The figure shows three views and two pictorial views of one solid part (mm, origin at its lowest corner). Answer the questions. Coordinates: 2 decimals unless noted, no trailing zeros. Order: outer loops, then holes, each group sorted by start corner. A loop starts at its lowest first (then second) coordinate and runs counter-clockwise, first axis right, second up.
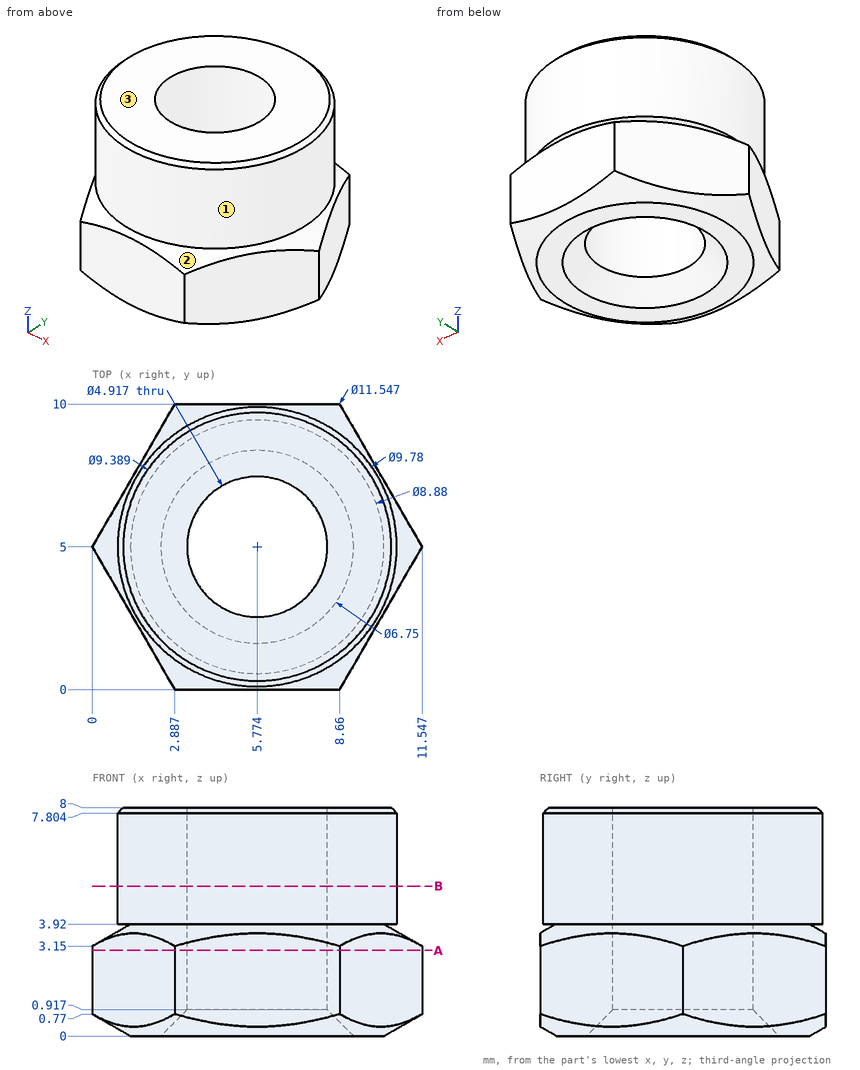
1) Straight lines are drawn through the part: probe 1 along X at (y, z) = (5.75, 3.5) (1 decimal); probe 2 along Y at (x, z) = (5, 3.5) (1 decimal); probe 3 along Y at (x, z) = (6.25, 4.5). For each, find the intervals that lie inside material, in ascending order.
2) A cutting plane is placed at A-A, the plane z = 3. Write down the section's boundary in (x, y).
3) The mould has two halves that part along Z. Classify the marked faces 1, 2 and 3: released by +Z, released by -Z, zero draft, split by the parting line, or undercut.
4) A cutting plane is placed at B-B, the plane z = 5.25. Write down the section's boundary in (x, y).
5) Each of these flat-tipped pins is pushed along its axis until it touches: P1, Ø4, axis at x = 5.77, y = 5, coming from the +Z side; P2, Ø1.5, axis at x = 6, z = 6, coming from the +Y side. Where does it stop, or does it pass through?
Working result:
1. probe 1: x = 0.7 to 3.4, 8.1 to 10.9
1. probe 2: y = 0 to 2.7, 7.3 to 10
1. probe 3: y = 0.13 to 2.59, 7.41 to 9.87
2. outline: (0, 5) - (2.89, 0) - (8.66, 0) - (11.55, 5) - (8.66, 10) - (2.89, 10) - close; hole circle Ø4.92 at (5.77, 5)
3. face 1: zero draft
3. face 2: undercut
3. face 3: released by +Z
4. outline: circle Ø9.78 at (5.77, 5); hole circle Ø4.92 at (5.77, 5)
5. P1: passes through
5. P2: stops at y = 9.89
